For this review, take the finished solid that the model builds, in its own axes (mm). Coordinates: 2 decimals unless noted, no trailing zeros. Loops run counter-clockwise (first coordinate to the right, second up) from the corner with the lowest first, then second, coordinate; pieces in that order, holes last. Notation, with made-up numbers: M 19,63 L 74,63 A31 cw 74,93 Z; hole C -38.5,59.25 d8. An arc over 180 degrees is marked long. Write item = value, one per line.
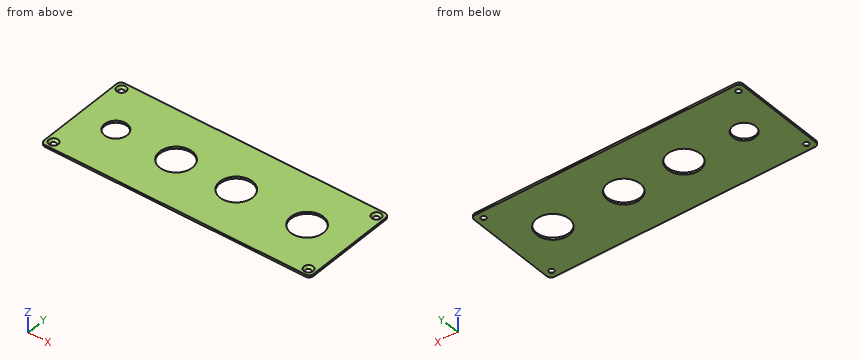
from build123d import *

# Parameters (mm, degrees)
SKETCH_1_W               = 190
SKETCH_1_H               = 70
EXTRUDE_1_DEPTH          = 1.5
FILLET_1_R               = 3
SKETCH_2_R               = 11.5
SKETCH_2_R_2             = 8
CUT_EXTRUDE_1_DEPTH      = 1.5
HOLE_WIZARD_1_AT_2_COUNT = 2
HOLE_WIZARD_1_AT_2_PITCH = 60
HOLE_WIZARD_1_AT_3_COUNT = 2
HOLE_WIZARD_1_AT_3_PITCH = 189.73665961
HOLE_WIZARD_1_AT_4_COUNT = 2
HOLE_WIZARD_1_AT_4_PITCH = 180


with BuildPart() as part:
    # 草图1 → 凸台-拉伸1 (new body)
    with BuildSketch(Plane.XY):
        Rectangle(SKETCH_1_W, SKETCH_1_H)
    extrude(amount=EXTRUDE_1_DEPTH)

    # 圆角1
    fillet_1_edges = [part.edges().sort_by_distance(p)[0] for p in [
        (95, -35, 0.75),
        (-95, -35, 0.75),
        (-95, 35, 0.75),
        (95, 35, 0.75),
    ]]
    fillet(fillet_1_edges, radius=FILLET_1_R)

    # 草图2 → 切除-拉伸1 (cut)
    with BuildSketch(Plane.XY.offset(1.5)):
        with Locations((15, 0)):
            Circle(SKETCH_2_R)
        with Locations((-27.5, 0)):
            Circle(SKETCH_2_R)
        with Locations((65, 0)):
            Circle(SKETCH_2_R)
        with Locations((-70, 0)):
            Circle(SKETCH_2_R_2)
    extrude(amount=-CUT_EXTRUDE_1_DEPTH, mode=Mode.SUBTRACT)

    # 草图4 → 打孔尺寸根据十字槽半沉头木螺钉的类型1 (revolve, cut)
    with BuildSketch(Plane(origin=(-90, 30, 1.5), x_dir=(0, -1, 0), z_dir=(1, 0, 0))):
        Polygon((0, 0), (0, 1.5), (1.7, 1.5), (1.7, 1.6), (3.3, 0), align=None)
    hole_wizard_1 = revolve(axis=Axis((-90, 30, 7.85), (0, 0, -1)), mode=Mode.SUBTRACT)

    # 打孔尺寸根据十字槽半沉头木螺钉的类型1 at 2: 打孔尺寸根据十字槽半沉头木螺钉的类型1 ×2
    with Locations(*[(0, -i * HOLE_WIZARD_1_AT_2_PITCH, 0) for i in range(1, HOLE_WIZARD_1_AT_2_COUNT)]):
        add(hole_wizard_1, mode=Mode.SUBTRACT)

    # 打孔尺寸根据十字槽半沉头木螺钉的类型1 at 3: 打孔尺寸根据十字槽半沉头木螺钉的类型1 ×2
    with Locations(*[Vector(0.9486832980505139, -0.3162277660168379, 0) * (i * HOLE_WIZARD_1_AT_3_PITCH) for i in range(1, HOLE_WIZARD_1_AT_3_COUNT)]):
        add(hole_wizard_1, mode=Mode.SUBTRACT)

    # 打孔尺寸根据十字槽半沉头木螺钉的类型1 at 4: 打孔尺寸根据十字槽半沉头木螺钉的类型1 ×2
    with Locations(*[(i * HOLE_WIZARD_1_AT_4_PITCH, 0, 0) for i in range(1, HOLE_WIZARD_1_AT_4_COUNT)]):
        add(hole_wizard_1, mode=Mode.SUBTRACT)


solid = part.part
Q1. For line 1 along Y through (x, z) = (-70, 1.2); line 2 along Y through (x, z) = (-27.5, 0.9); line 3 along X through (y, z) = (-2, 0.6), list the stretches that pass through material, from the lowest coordinate up.
Solved:
line_1 = -35 to -8, 8 to 35
line_2 = -35 to -11.5, 11.5 to 35
line_3 = -95 to -77.75, -62.25 to -38.82, -16.18 to 3.68, 26.32 to 53.68, 76.32 to 95
Q2. For pin 1 Ø18.5 at (x, y) = (-27.5, 0) entering from -Z; pin 2 Ø10 at (x, y) = (-35, -19) entering from -Z, all flat-tipped, find the tip position at first contact; note any pin that passes through.
Solved:
pin_1 = through
pin_2 = 0
Q3. Add section A-A (x = 90). Write out the cut boundary in (y, z), and give its area (3 significant figures).
Solved:
outline = M -35,0 L -31.8,0 L -33.3,1.5 L -35,1.5 Z; M -28.2,0 L 28.2,0 L 26.7,1.5 L -26.7,1.5 Z; M 31.8,0 L 35,0 L 35,1.5 L 33.3,1.5 Z
area = 89.7 mm²
Q4. Add section B-B (y = 30). Write out the cut boundary in (x, z), and give its area (3 significant figures).
Solved:
outline = M -95,0 L -91.8,0 L -93.3,1.5 L -95,1.5 Z; M -88.2,0 L 88.2,0 L 86.7,1.5 L -86.7,1.5 Z; M 91.8,0 L 95,0 L 95,1.5 L 93.3,1.5 Z
area = 270 mm²
Q5. Add section D-D (x = 65). Write out the cut boundary in (y, z), and give its area (3 significant figures).
Solved:
outline = M -35,0 L -11.5,0 L -11.5,1.5 L -35,1.5 Z; M 11.5,0 L 35,0 L 35,1.5 L 11.5,1.5 Z
area = 70.5 mm²
Q6. Add section C-C (y = 0). Write out the cut boundary in (x, z).
Solved:
outline = M -95,0 L -78,0 L -78,1.5 L -95,1.5 Z; M -62,0 L -39,0 L -39,1.5 L -62,1.5 Z; M -16,0 L 3.5,0 L 3.5,1.5 L -16,1.5 Z; M 26.5,0 L 53.5,0 L 53.5,1.5 L 26.5,1.5 Z; M 76.5,0 L 95,0 L 95,1.5 L 76.5,1.5 Z
